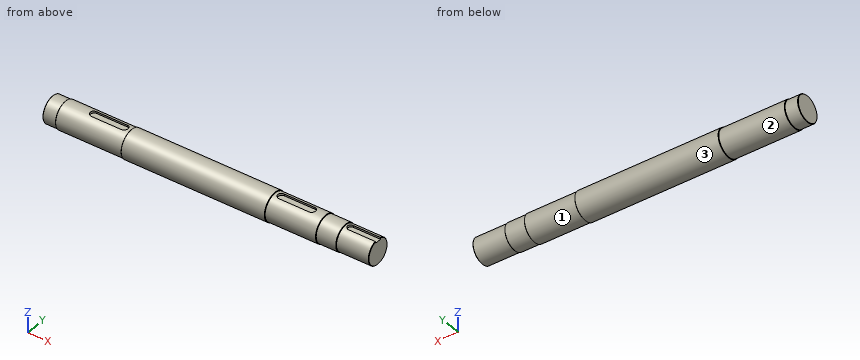
```python
from build123d import *

# Parameters (mm, degrees)
CUT_EXTRUDE1_DEPTH = 12
CUT_EXTRUDE2_DEPTH = 12
CHAMFER1_SIZE      = 2


with BuildPart() as part:
    # Sketch1 → Revolve1 (revolve)
    with BuildSketch(Plane.XY, mode=Mode.PRIVATE) as revolve1_sk:
        Polygon((-796, 70), (-728, 70), (-728, 72.5), (-380, 72.5), (-380, 75), (380, 75), (380, 72.5), (648, 72.5), (648, 70), (753, 70), (753, 67.5), (923, 67.5), (923, 0), (-796, 0), align=None)
    revolve(revolve1_sk.sketch.rotate(Axis((-820.662631097, 0, 0), (1, 0, 0)), 90), axis=Axis((-820.662631097, 0, 0), (1, 0, 0)))

    # Sketch2 → Cut-Extrude1 (cut)
    with BuildSketch(Plane.XY.offset(67.5)):
        with BuildLine():
            Line((923, -18), (781, -18))
            ThreePointArc((781, -18), (763, 0), (781, 18))
            Line((781, 18), (923, 18))
            Line((923, 18), (923, 0))
            Line((923, 0), (923, -18))
        make_face()
    extrude(amount=-CUT_EXTRUDE1_DEPTH, mode=Mode.SUBTRACT)

    # Sketch3 → Cut-Extrude2 (cut)
    with BuildSketch(Plane.XY.offset(72.5)):
        with BuildLine():
            Line((-575, -20), (-415, -20))
            ThreePointArc((-415, -20), (-395, 0), (-415, 20))
            Line((-415, 20), (-575, 20))
            ThreePointArc((-575, 20), (-595, 0), (-575, -20))
        make_face()
        with BuildLine():
            Line((575, 20), (415, 20))
            ThreePointArc((415, 20), (395, 0), (415, -20))
            Line((415, -20), (575, -20))
            ThreePointArc((575, -20), (595, 0), (575, 20))
        make_face()
    extrude(amount=-CUT_EXTRUDE2_DEPTH, mode=Mode.SUBTRACT)

    # Chamfer1
    chamfer1_edges = [part.edges().sort_by_distance(p)[0] for p in [
        (-796, 0, -70),
        (-728, 0, -72.5),
        (-380, 0, -75),
        (380, 0, -75),
        (648, 0, -72.5),
        (753, 0, -70),
        (923, 0, -67.5),
    ]]
    chamfer(chamfer1_edges, length=CHAMFER1_SIZE)


solid = part.part
```
Read the model definition and answer for the solid it produces. Units are mm, in the model's axes. Face numbers are marked on the shaded views. A direction names the side the tool comes from. Coordinates: 2 decimals unless noted, no trailing zeros. Write each loop counter-clockwise with the first axis right and the second up, starting at its lowest first coordinate (ties: lowest second). Pieces come first, ordered by that corner, then holes. Notation, with made-up numbers: (80, 40) -> (109, 40) arc R18 ccw to (109, 66) -> close; hole circle Ø4 at (59.25, -6.5). An arc over 180 degrees is marked (long way). Return JSON: item names as keys, results as strings.
1. Find the intervals of material crossed by line 1 along Z through (x, y) = (66, 1.5) (3 decimals); line 2 along Y through (x, z) = (562, 1); line 3 along Y through (x, z) = (164, -7), in increasing order. Write a range as from..to.
Found:
{"line 1": "-74.985..74.985", "line 2": "-72.49..72.49", "line 3": "-74.67..74.67"}
2. A cutting plane is placed at A-A (x = -247.5). Determine the outline of the cut face in (y, z), and give its area (3 significant figures).
Found:
{"outline": "circle Ø150 at (0, 0)", "area": "17,700 mm2"}
3. Each of these flat-tipped pins is pushed along its axis until it touches: P1, Ø2, axis at x = -495, z = 46.5, coming from the -Y side; P2, Ø1.5, axis at x = 417, z = 38.5, coming from the -Y side; P3, Ø7.5, axis at x = -490, z = 65.5, coming from the +Y side. Where does it stop, or does it pass through?
Found:
{"P1": "y = -56.44", "P2": "y = -61.9", "P3": "y = 37.99"}
4. A tool of negligible diameter and unlimited length cuts with its end or side. For the marked faces 1, 2 and 3, from which of +Z, -Z, +X, -X, +Y, -Y can it reach the whole face along a straight path? Write none if from no direction.
Found:
{"face 1": "+X", "face 2": "-X", "face 3": "+X, -X"}
